Can you work these out from the drawing? Everything is in mm from the part's minimum corner. Round coordinates to 2 decimals unless told otherwise and drop trailing zeros. Write each loop counter-clockwise with the first axis right and the second up, starting at its lowest first coordinate (ties: lowest second). Pieces come first, ordered by that corner, then holes. Notation, with made-up numbers: (76.5, 55.25) - (99.5, 55.25) arc R20 cw to (99.5, 72.25) - close; hole circle Ø1 at (38.25, 74.25). An arc over 180 degrees is marked (long way). One line per item, written item: value. Start each with the question number.
Item 1: Imagine slicing it at C-C, the plane x = 30.5. Please give me the cut outline in (y, z) (1 decimal).
Item 2: Imagine slicing it at D-D, the plane x = 4.5. Please give me the cut outline in (y, z).
Item 3: Imagine slicing it at A-A, the plane y = 17. Please give me the cut outline in (x, z).
Item 4: Thinking about a two-plate mould opening in Y: for the marked faces 1, 2 and 3, which applies, released by +Y, released by -Y, zero draft, split by the parting line, or undercut?
Item 5: Imagine slicing it at B-B, the plane z = 5. Please give me the cut outline in (x, y) (1 decimal).
Item 6: If I drill on line 1 (Y direction, x = 15, z = 4.25) (1 decimal); line 2 (Y direction, x = 22.5, z = 10.5); line 3 (X direction, y = 19, z = 11.5) (1 decimal), over which ranges is the centre line in solid material (lowest first)?
Item 7: For P1, Ø2, axis at x = 22, z = 12, coming from the -Y side; P2, Ø2, axis at y = 14, z = 10.5, coming from the +X side; P3, Ø3, axis at x = 16.5, z = 8, coming from the -Y side, each with a flat end and sliding along its axis, tell me the tip position at first contact or that it passes through.
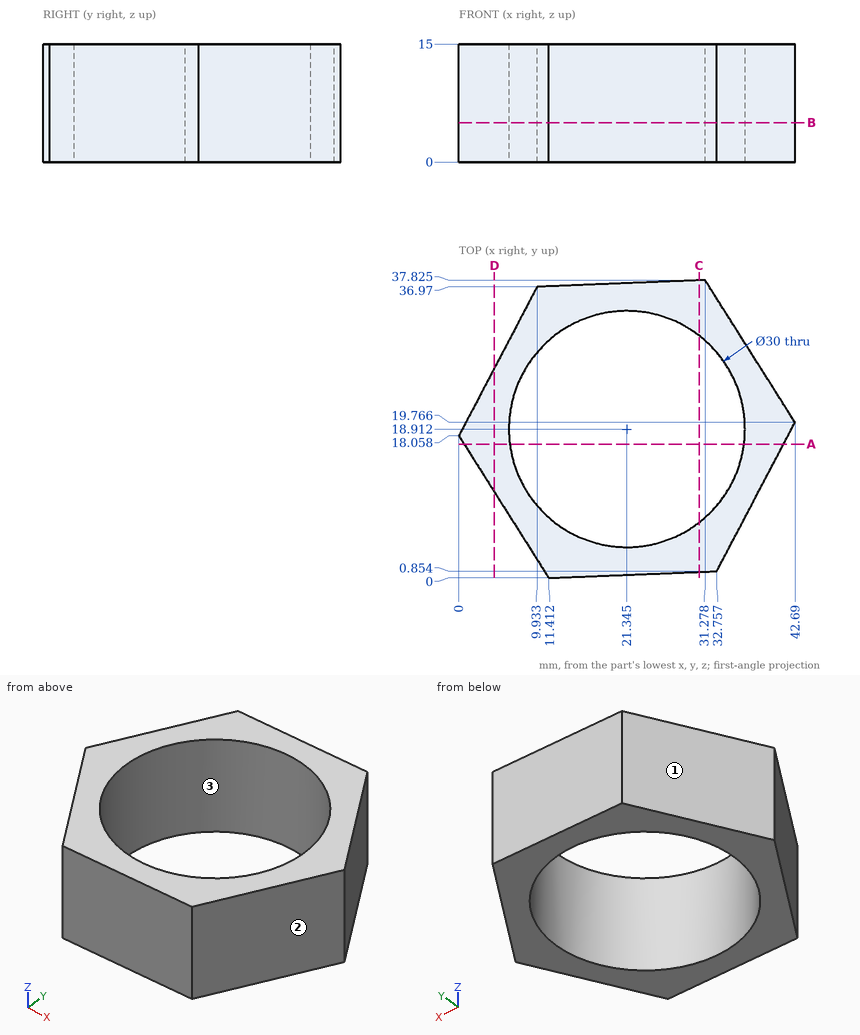
Values follow:
1. outline: (0.8, 0) - (7, 0) - (7, 15) - (0.8, 15) - close; (30.8, 0) - (37.8, 0) - (37.8, 15) - (30.8, 15) - close
2. outline: (10.94, 0) - (26.63, 0) - (26.63, 15) - (10.94, 15) - close
3. outline: (0.67, 0) - (6.47, 0) - (6.47, 15) - (0.67, 15) - close; (36.22, 0) - (41.24, 0) - (41.24, 15) - (36.22, 15) - close
4. face 1: released by +Y
4. face 2: released by -Y
4. face 3: undercut
5. outline: (0, 18.1) - (11.4, 0) - (32.8, 0.9) - (42.7, 19.8) - (31.3, 37.8) - (9.9, 37) - close; hole circle Ø30 at (21.3, 18.9)
6. line 1: y = 0.1 to 5.3, 32.5 to 37.2
6. line 2: y = 0.44 to 3.96, 33.87 to 37.47
6. line 3: x = 0.5 to 6.3, 36.3 to 42.3
7. P1: stops at y = 0.38
7. P2: stops at x = 40.19
7. P3: stops at y = 0.14
